```python
from build123d import *

# Parameters (mm, degrees)
BOSS_EXTRUDE1_DEPTH   = 10
SKETCH2_R             = 6
BOSS_EXTRUDE2_DEPTH   = 260
M5_TAPPED_HOLE1_D     = 4.2
M5_TAPPED_HOLE1_DEPTH = 36.9
M5_TAPPED_HOLE1_TIP   = 1.2618073
CUT_EXTRUDE1_DEPTH    = 266.047165614
CHAMFER1_SIZE         = 3


with BuildPart() as part:
    # Sketch1 → Boss-Extrude1 (new body)
    with BuildSketch(Plane(origin=(0, 0, 0), x_dir=(1, 0, 0), z_dir=(0, 1, 0))):
        Polygon((-25, 25), (-5, 45), (5, 45), (25, 25), (25, -25), (-25, -25), align=None)
    extrude(amount=BOSS_EXTRUDE1_DEPTH)

    # Sketch2 → Boss-Extrude2 (add)
    with BuildSketch(Plane.XZ):
        with Locations(Location((0, -30, 0), (0, 0, 90))):
            Circle(SKETCH2_R)
    extrude(amount=BOSS_EXTRUDE2_DEPTH)

    # M5 Tapped Hole1
    with Locations(Plane(origin=(0, 0, -45), x_dir=(-1, 0, 0), z_dir=(0, 0, -1))):
        with Locations((0, 5)):
            Hole(M5_TAPPED_HOLE1_D / 2, depth=M5_TAPPED_HOLE1_DEPTH)
            with Locations((0, 0, -(M5_TAPPED_HOLE1_DEPTH + M5_TAPPED_HOLE1_TIP / 2))):  # 118° drill point
                Cone(0, M5_TAPPED_HOLE1_D / 2, M5_TAPPED_HOLE1_TIP, mode=Mode.SUBTRACT)

    # Sketch5 → Cut-Extrude1 (cut, through all)
    with BuildSketch(Plane.XZ):
        with BuildLine():
            Line((3, 10), (3, -10))
            ThreePointArc((3, -10), (0, -13), (-3, -10))
            Line((-3, -10), (-3, 10))
            ThreePointArc((-3, 10), (0, 13), (3, 10))
        make_face()
    extrude(amount=-CUT_EXTRUDE1_DEPTH, mode=Mode.SUBTRACT)

    # Chamfer1
    chamfer1_edges = [part.edges().sort_by_distance(p)[0] for p in [
        (25, 5, 25),
        (-25, 5, 25),
    ]]
    chamfer(chamfer1_edges, length=CHAMFER1_SIZE)


solid = part.part
```
Source: CAD feature listing. Evaluate the final solid. Frame: model axes, mm. A direction names the side the tool comes from. Give positions to 0.01 mm unless a question says otherwise; leave off trailing zeros. Loops run counter-clockwise (first coordinate to the right, second up) from the corner with the lowest first, then second, coordinate; pieces in that order, holes last. Notation, with made-up numbers: (23, -18) - (60, -18) arc R21 ccw to (60, -3) - close; hole circle Ø1 at (76.5, 63.5). An arc over 180 degrees is marked (long way). Use CSV: the item, a comma, the result in double quotes.
1) Cut plane C-C (x = -17). Output: boundary loops of the cut face in (y, z), and give its area (3 significant figures).
Worked out:
outline,"(0, -33) - (10, -33) - (10, 25) - (0, 25) - close"
area,"580 mm^2"
2) Line query: line 1 (Y direction, x = 0, z = -26); line 2 (Y direction, x = 0, z = -18.5); line 3 (X direction, y = 5, z = -28). Output: solid intervals per line, ascending.
Worked out:
line 1,"y = -260 to 2.9, 7.1 to 10"
line 2,"y = 0 to 2.9, 7.1 to 10"
line 3,"x = -22 to -2.1, 2.1 to 22"
3) Cut plane B-B (z = -4). Output: boundary loops of the cut face in (x, y), and give its area (3 significant figures).
Worked out:
outline,"(-25, 0) - (-3, 0) - (-3, 10) - (-25, 10) - close; (3, 0) - (25, 0) - (25, 10) - (3, 10) - close"
area,"440 mm^2"
4) Cut plane A-A (z = -30). Output: boundary loops of the cut face in (x, y).
Worked out:
outline,"(-20, 0) - (-6, 0) - (-6, -260) - (6, -260) - (6, 0) - (20, 0) - (20, 10) - (-20, 10) - close; hole circle Ø4.2 at (0, 5)"
5) Pin query (flat end, axial travel): P1, Ø1.5, axis at y = -158, z = -29, coming from the -X side; P2, Ø6, axis at y = -99, z = -35, coming from the -X side; P3, Ø5, axis at x = -5, y = -58.5, coming from the +Z side. Return the tip coordinate at first contact, or that it passes through.
Worked out:
P1,"stops at x = -5.99"
P2,"stops at x = -5.66"
P3,"stops at z = -24.55"
6) Cut plane D-D (y = -149). Output: boundary loops of the cut face in (x, z).
Worked out:
outline,"circle Ø12 at (0, -30)"
7) Set-up query: faces 1 (the flat face through (6, 10, -10)), 2 (the cylindrical face through (0, -128, -36)), 3 (the flat face through (-3, 5, 0)). Return all of +Z, -Z, +X, -X, +Y, -Y with unobstructed straight access to the full face (end or side cutting, diameter ignored); none if empty.
Worked out:
face 1,"+Z, -Z, +X, -X, +Y"
face 2,"-Y"
face 3,"+Y, -Y"
